```python
from build123d import *

# Parameters (mm, degrees)
SKETCH1_W                                           = 35
SKETCH1_H                                           = 30
BOSS_EXTRUDE1_DEPTH                                 = 15
CBORE_FOR_M4_HEX_SOCKET_HEAD_CAP_SCREW1_D           = 4.5
CBORE_FOR_M4_HEX_SOCKET_HEAD_CAP_SCREW1_CBORE_D     = 8
CBORE_FOR_M4_HEX_SOCKET_HEAD_CAP_SCREW1_CBORE_DEPTH = 4.4
M8_TAPPED_HOLE1_D                                   = 6.8
M8_TAPPED_HOLE1_DEPTH                               = 22.25
M8_TAPPED_HOLE1_TIP                                 = 2.042926105
CHAMFER1_SIZE                                       = 2


with BuildPart() as part:
    # Sketch1 → Boss-Extrude1 (new body)
    with BuildSketch(Plane.XY):
        Rectangle(SKETCH1_W, SKETCH1_H)
    extrude(amount=BOSS_EXTRUDE1_DEPTH)

    # CBORE for M4 Hex Socket Head Cap Screw1 (through all)
    with Locations(Plane(origin=(0, 15, 0), x_dir=(1, 0, 0), z_dir=(0, 1, 0))):
        with Locations((-10, -7.5), (10, -7.5)):
            CounterBoreHole(CBORE_FOR_M4_HEX_SOCKET_HEAD_CAP_SCREW1_D / 2, CBORE_FOR_M4_HEX_SOCKET_HEAD_CAP_SCREW1_CBORE_D / 2, CBORE_FOR_M4_HEX_SOCKET_HEAD_CAP_SCREW1_CBORE_DEPTH)

    # M8 Tapped Hole1
    with Locations(Plane.XY.offset(15)):
        with Locations((0, 7)):
            Hole(M8_TAPPED_HOLE1_D / 2, depth=M8_TAPPED_HOLE1_DEPTH)
            with Locations((0, 0, -(M8_TAPPED_HOLE1_DEPTH + M8_TAPPED_HOLE1_TIP / 2))):  # 118° drill point
                Cone(0, M8_TAPPED_HOLE1_D / 2, M8_TAPPED_HOLE1_TIP, mode=Mode.SUBTRACT)

    # Chamfer1
    chamfer1_edges = [part.edges().sort_by_distance(p)[0] for p in [
        (17.5, -15, 7.5),
        (-17.5, -15, 7.5),
        (-17.5, 15, 7.5),
        (17.5, 15, 7.5),
    ]]
    chamfer(chamfer1_edges, length=CHAMFER1_SIZE)


solid = part.part
```
CAD build for the part. Positions are in the model's coordinates, mm. A direction names the side the tool comes from. Give positions to 0.01 mm unless a question says otherwise; leave off trailing zeros. Order: outer loops, then holes, each group sorted by start corner. A loop starts at its lowest first (then second) coordinate and runs counter-clockwise, first axis right, second up. Notation, with made-up numbers: M -17.5,65 L 9.5,65 A27 ccw 9.5,82 Z; hole C 69.25,80 d11. An arc over 180 degrees is marked long. Put each result on its own line as item: value. Start each with the question number.
(1) Which spindle directions (+Z, -Z, +X, -X, +Y, -Y) get a long thin tool onto all of the face, cutting with end or side? Do faces 5 (the flat face through (17.5, 0, 7)), 6 (the flat face through (-8, 10.6, 9)). Say none if no direction does.
(2) Drill centre lines: line 1 along Z through (x, y) = (-10, 12.4); line 2 along Y through (x, z) = (0, 6.25); line 3 along Z through (x, y) = (-10, -4.5). Where is each one in solid material? Low to high.
(3) Saw through at C-C, the plane z = 7.5. Write the cut outline in (x, y), then the cut area to 3 significant figures.
(4) Saw through at D-D, the plane x = -10. Write the cut outline in (y, z), then the cut area to 3 significant figures.
(5) Saw through at A-A, the plane x = 0. Write the cut outline in (y, z), then the cut area to 3 significant figures.
(6) Saw through at B-B, the plane y = 7. Write the cut outline in (x, z), then the cut area to 3 significant figures.
(7) Mould opens along Y. For faces 1 (the cylindrical face through (0.74, 3.68, 7.4)), 2 (the flat face through (-17.5, 0, 7)), 3 (the flat face through (-16.5, -14, 7.4)), 4 (the flat face through (16.5, 14, 7.4)) say: +Y half, -Y half, draft (parallel to the pull), parting line (faces both ways), or undercut.
(8) Flat gauge pins, fed straight in: pin 1 Ø4 at (x, y) = (0, 7) entering from -Z; pin 2 Ø9 at (x, z) = (8, 9) entering from +Y; pin 3 Ø5 at (x, z) = (-10, 7.5) entering from +Y. Where does each tip first touch, or does it go through?
Check result:
1. face 5: +Z, -Z, +X, +Y, -Y
1. face 6: +Y
2. line 1: z = 0 to 3.5, 11.5 to 15
2. line 2: y = -15 to 3.6, 10.4 to 15
2. line 3: z = 0 to 5.25, 9.75 to 15
3. outline: M -17.5,-13 L -15.5,-15 L -12.25,-15 L -12.25,10.6 L -14,10.6 L -14,15 L -15.5,15 L -17.5,13 Z; M -7.75,-15 L 7.75,-15 L 7.75,10.6 L 6,10.6 L 6,15 L -6,15 L -6,10.6 L -7.75,10.6 Z; M 12.25,-15 L 15.5,-15 L 17.5,-13 L 17.5,13 L 15.5,15 L 14,15 L 14,10.6 L 12.25,10.6 Z; hole C 0,7 d6.8
3. area: 705 mm2
4. outline: M -15,0 L 15,0 L 15,3.5 L 10.6,3.5 L 10.6,5.25 L -15,5.25 Z; M -15,9.75 L 10.6,9.75 L 10.6,11.5 L 15,11.5 L 15,15 L -15,15 Z
4. area: 300 mm2
5. outline: M -15,0 L 3.6,0 L 3.6,15 L -15,15 Z; M 10.4,0 L 15,0 L 15,15 L 10.4,15 Z
5. area: 348 mm2
6. outline: M -17.5,0 L -3.4,0 L -3.4,15 L -17.5,15 Z; M 3.4,0 L 17.5,0 L 17.5,15 L 3.4,15 Z; hole C -10,7.5 d4.5; hole C 10,7.5 d4.5
6. area: 391 mm2
7. face 1: undercut
7. face 2: draft
7. face 3: -Y half
7. face 4: +Y half
8. pin 1: passes through
8. pin 2: stops at y = 15
8. pin 3: stops at y = 10.6
